```python
from build123d import *

# Parameters (mm, degrees)
EXTRUDE_THIN1_DEPTH     = 12.7
SKETCH3_W               = 22.8
SKETCH3_H               = 18.7
BOSS_EXTRUDE2_DEPTH     = 2
FILLET1_R               = 2
SKETCH4_R               = 1.25
CUT_EXTRUDE1_DEPTH      = 2
CUT_EXTRUDE2_DEPTH      = 61.42253709
CUT_EXTRUDE2_DEPTH_BACK = 61.42253709
SKETCH5_R               = 2.75
SKETCH6_R               = 1.25
CUT_EXTRUDE3_DEPTH      = 10
CUT_EXTRUDE4_DEPTH      = 131.301684531
CUT_EXTRUDE4_DEPTH_BACK = 131.301684531
SKETCH7_W               = 21.210036283
SKETCH7_H               = 32.49756926


with BuildPart() as part:
    # Sketch1 → Extrude-Thin1 (new body)
    with BuildSketch(Plane.XY):
        Polygon((51.165574182, 84.975681723), (42.185318061, 93.955937844), (42.185318061, 113.634045339), (40.185318061, 113.634045339), (40.185318061, 93.127510719), (49.75136062, 83.561468161), align=None)
    extrude(amount=-EXTRUDE_THIN1_DEPTH)

    # Sketch5 → Cut-Extrude2 (cut, two sides: drawn at the far end of the back side and taken through both)
    with BuildSketch(Plane(origin=(68.070627953, 68.070627953, 0), x_dir=(0, 0, -1), z_dir=(0.7071067811865513, 0.7071067811865437, 0)).offset(-CUT_EXTRUDE2_DEPTH_BACK)):
        with Locations(Location((6.35, 30.257356315, 0), (0, 0, 90))):
            Circle(SKETCH5_R)
    extrude(amount=CUT_EXTRUDE2_DEPTH + CUT_EXTRUDE2_DEPTH_BACK, mode=Mode.SUBTRACT)

    # Sketch6 → Cut-Extrude3 (cut)
    with BuildSketch(Plane(origin=(66.65641439, 66.65641439, 0), x_dir=(0, 0, 1), z_dir=(-0.7071067811865513, -0.7071067811865437, 0))):
        with Locations(Location((-10.65, 34.557356315, 0), (0, 0, 270))):
            Circle(SKETCH6_R)
        with Locations(Location((-2.05, 34.557356315, 0), (0, 0, 270))):
            Circle(SKETCH6_R)
        with Locations(Location((-2.05, 25.957356315, 0), (0, 0, 270))):
            Circle(SKETCH6_R)
        with Locations(Location((-10.65, 25.957356315, 0), (0, 0, 270))):
            Circle(SKETCH6_R)
    extrude(amount=-CUT_EXTRUDE3_DEPTH, mode=Mode.SUBTRACT)

    # Sketch7 → Cut-Extrude4 (cut, two sides: drawn at the far end of the back side and taken through both)
    with BuildSketch(Plane.XY.offset(3).offset(-CUT_EXTRUDE4_DEPTH_BACK)):
        with Locations((44.470427981, 97.385260709)):
            Rectangle(SKETCH7_W, SKETCH7_H)
    extrude(amount=CUT_EXTRUDE4_DEPTH + CUT_EXTRUDE4_DEPTH_BACK, mode=Mode.SUBTRACT)


with BuildPart() as body_2:
    # Sketch3 → Boss-Extrude2 (new body)
    with BuildSketch(Plane(origin=(0, 113.634045339, 0), x_dir=(1, 0, 0), z_dir=(0, 1, 0))):
        with Locations((45.675446122, 6.35)):
            Rectangle(SKETCH3_W, SKETCH3_H)
    extrude(amount=BOSS_EXTRUDE2_DEPTH)

    # Fillet1
    fillet1_edges = [body_2.edges().sort_by_distance(p)[0] for p in [
        (57.075446122, 114.634045339, 3),
        (34.275446122, 114.634045339, 3),
        (34.275446122, 114.634045339, -15.7),
        (57.075446122, 114.634045339, -15.7),
    ]]
    fillet(fillet1_edges, radius=FILLET1_R)

    # Sketch4 → Cut-Extrude1 (cut)
    with BuildSketch(Plane(origin=(0, 115.634045339, 0), x_dir=(1, 0, 0), z_dir=(0, 1, 0))):
        with Locations(Location((55.075446122, 13.7, 0), (0, 0, 270))):
            Circle(SKETCH4_R)
        with Locations(Location((55.075446122, -1, 0), (0, 0, 270))):
            Circle(SKETCH4_R)
        with Locations(Location((36.275446122, -1, 0), (0, 0, 270))):
            Circle(SKETCH4_R)
        with Locations(Location((36.275446122, 13.7, 0), (0, 0, 270))):
            Circle(SKETCH4_R)
    extrude(amount=-CUT_EXTRUDE1_DEPTH, mode=Mode.SUBTRACT)


solid = body_2.part
```
The model under review builds one solid part; all positions refer to its coordinate system, in mm. Round coordinates to 2 decimals unless told otherwise and drop trailing zeros. Write each loop counter-clockwise with the first axis right and the second up, starting at its lowest first coordinate (ties: lowest second). Pieces come first, ordered by that corner, then holes. Notation, with made-up numbers: M -32,17.5 L 17,17.5 A11 cw 17,35.5 Z; hole C 54,83 d11. An arc over 180 degrees is marked long. Use CSV: the item, a comma, the result in double quotes. Start each with the question number.
(1) We need section C-C, the plane z = 1.25. State the section outline as (x, y) points, then the cut area to 3 significant figures.
(2) For line 1 along X through (y, z) = (114.4, -13.7); line 2 along Z through (x, y) = (55, 115.25); line 3 along X through (y, z) = (113.85, 0.25), list the stretches that pass through material, from the lowest coordinate up.
(3) We need section B-B, the plane x = 36.75. State the section outline as (y, z) points.
(4) We need section A-A, the plane y = 114.4. State the section outline as (x, z) points, then the cut area to 3 significant figures.
(5) The part is to be moulded in two halves that separate along X. For faces 1 (the face through (34.846, 114.648, -15.099)), 2 (the face through (37.515, 114.648, -13.863)), 3 (the face through (46, 115, -15.7)), say which applies: +X half, -X half, draft (parallel to the pull), parting line (faces both ways), or undercut.
Findings:
1,outline,"M 34.29,113.63 L 35.05,113.63 L 35.05,115.63 L 34.29,115.63 Z; M 37.5,113.63 L 53.85,113.63 L 53.85,115.63 L 37.5,115.63 Z; M 56.3,113.63 L 57.06,113.63 L 57.06,115.63 L 56.3,115.63 Z"
1,area,"35.7 mm^2"
2,line 1,"34.28 to 35.03, 37.53 to 53.83, 56.33 to 57.08"
2,line 2,"-15.7 to -14.95, -12.45 to -0.25, 2.25 to 3"
2,line 3,"34.28 to 35.28, 37.28 to 54.08, 56.08 to 57.08"
3,outline,"M 113.63,-15.7 L 115.63,-15.7 L 115.63,-14.86 L 113.63,-14.86 Z; M 113.63,-12.54 L 115.63,-12.54 L 115.63,-0.16 L 113.63,-0.16 Z; M 113.63,2.16 L 115.63,2.16 L 115.63,3 L 113.63,3 Z"
4,outline,"M 34.28,-13.7 A2 ccw 36.28,-15.7 L 55.08,-15.7 A2 ccw 57.08,-13.7 L 57.08,1 A2 ccw 55.08,3 L 36.28,3 A2 ccw 34.28,1 Z; hole C 36.28,-13.7 d2.5; hole C 36.28,1 d2.5; hole C 55.08,-13.7 d2.5; hole C 55.08,1 d2.5"
4,area,"403 mm^2"
5,face 1,"-X half"
5,face 2,"undercut"
5,face 3,"draft"
